from build123d import *

# Parameters (mm, degrees)
SKETCH_1_W                   = 60
SKETCH_1_H                   = 35
EXTRUDE_1_DEPTH              = 5
SKETCH_2_R                   = 2.25
CUT_EXTRUDE_1_DEPTH          = 37.142080737
CUT_EXTRUDE_2_DEPTH          = 37.142080737
SKETCH_5_W                   = 80
SKETCH_5_H                   = 50
EXTRUDE_3_DEPTH              = 10
HOLE_WIZARD_M4_1_D           = 4.5
HOLE_WIZARD_M4_1_CBORE_D     = 8
HOLE_WIZARD_M4_1_CBORE_DEPTH = 4.4
FILLET_1_R                   = 5


with BuildPart() as part:
    # 草图1 → 凸台-拉伸1 (new, symmetric)
    with BuildSketch(Plane(origin=(0, 0, 0), x_dir=(1, 0, 0), z_dir=(0, 1, 0))):
        Rectangle(SKETCH_1_W, SKETCH_1_H)
    extrude(amount=EXTRUDE_1_DEPTH, both=True)

    # 草图2 → 切除-拉伸1 (cut, through all)
    with BuildSketch(Plane.XZ.offset(5)):
        with Locations(Location((-15, 12.5, 0), (0, 0, 270))):
            Circle(SKETCH_2_R)
        with Locations(Location((-15, 2.5, 0), (0, 0, 270))):
            Circle(SKETCH_2_R)
    extrude(amount=-CUT_EXTRUDE_1_DEPTH, mode=Mode.SUBTRACT)

    # 草图3 → 切除-拉伸2 (cut, through all)
    with BuildSketch(Plane.XZ.offset(5)):
        with BuildLine():
            ThreePointArc((-27.188596105, 11.275), (-15, 0.25), (-2.811403895, 11.275))
            ThreePointArc((-2.811403895, 11.275), (-4.825125629, 13.738721733), (-7.288847362, 11.725))
            ThreePointArc((-7.288847362, 11.725), (-15, 4.75), (-22.711152638, 11.725))
            ThreePointArc((-22.711152638, 11.725), (-25.174874371, 13.738721733), (-27.188596105, 11.275))
        make_face()
    extrude(amount=-CUT_EXTRUDE_2_DEPTH, mode=Mode.SUBTRACT)

    # 草图5 → 凸台-拉伸3 (add)
    with BuildSketch(Plane(origin=(30, 0, 0), x_dir=(0, 0, -1), z_dir=(1, 0, 0))):
        Rectangle(SKETCH_5_W, SKETCH_5_H)
    extrude(amount=EXTRUDE_3_DEPTH)

    # M4 六角凹头螺钉的柱形沉头孔1 (through all)
    with Locations(Plane.ZY.offset(-30)):
        with Locations((30, 15), (-30, 15), (-30, -15), (30, -15)):
            CounterBoreHole(HOLE_WIZARD_M4_1_D / 2, HOLE_WIZARD_M4_1_CBORE_D / 2, HOLE_WIZARD_M4_1_CBORE_DEPTH)

    # 圆角1
    fillet_1_edges = [part.edges().sort_by_distance(p)[0] for p in [
        (35, -25, -40),
        (35, 25, -40),
        (35, 25, 40),
        (35, -25, 40),
        (-30, 0, 17.5),
        (-30, 0, -17.5),
    ]]
    fillet(fillet_1_edges, radius=FILLET_1_R)


solid = part.part
Verification items for the finished model (mm, model axes). A direction names the side the tool comes from. Coordinates: 2 decimals unless noted, no trailing zeros. Write each loop counter-clockwise with the first axis right and the second up, starting at its lowest first coordinate (ties: lowest second). Pieces come first, ordered by that corner, then holes. Notation, with made-up numbers: (34.5, 85) -> (81.5, 85) arc R16 cw to (81.5, 93) -> close; hole circle Ø8 at (68, 82). An arc over 180 degrees is marked (long way). One line per item, written item: value. Start each with the question number.
Q1. Thickness scan on L1, parallel to Y at x = 38.35, z = 30; L2, parallel to Y at x = 32.2, z = 30; L3, parallel to Z at x = 36, y = -13.5. Record the ranges inside material, lowest first. Write a range as from..to.
Q2. Cross-section at C-C on x = -15. Enter the section's corners in (y, z), and give its area (3 significant figures).
Q3. Cross-section at B-B on z = 30. Enter the section's corners in (x, y), and give its area (3 significant figures).
Q4. Cross-section at D-D on y = 4. Enter the section's corners in (x, z) (3 decimals), and give its area (3 significant figures).
Q5. Cross-section at A-A on y = -15. Enter the section's corners in (x, z), and give its area (3 significant figures).
Q6. Access from +Z, -Z, +X, -X, +Y, -Y to the whole of each face (thin tool, end or side, straight path). Record for faces 5 (the flat face through (34.4, 13, -28)), 6 (the cylindrical face through (-4.776, -0.07, 13.733)), 7 (the flat face through (0, -5, 0)), 8 (the flat face through (2, 0, 17.5)).
Q7. Mould release check, pull along Y, two halves, no side actions. Record for faces 1 (the flat face through (30, 6, 1)), 2 (the cylindrical face through (32.17, -12.3, 27.05)), 3 (the flat face through (35, -25, 0)), 4 (the cylindrical face through (32.169, 18.966, -30.521)): pulls with the +Y half, pulls with the -Y half, needs draft (parallel to the pull), parting line crosses it, or undercut.
Q8. Go/stop test with flat-tipped pins: P1, Ø6.5, axis at y = -15, z = 30, coming from the -X side; P2, Ø8, axis at x = 7.5, z = -18, coming from the +Y side; P3, Ø1, axis at y = 3.5, z = -22.5, coming from the -X side; P4, Ø2.5, axis at y = 15.5, z = 30.5, coming from the -X side. Record where each tip stops, or that it passes through.
Checked values:
1. L1: y = -25..-17.25, -12.75..12.75, 17.25..25
1. L2: y = -25..-19, -11..11, 19..25
1. L3: z = -40..-31.68, -28.32..28.32, 31.68..40
2. outline: (-5, -17.5) -> (5, -17.5) -> (5, 0.25) -> (-5, 0.25) -> close; (-5, 4.75) -> (5, 4.75) -> (5, 10.25) -> (-5, 10.25) -> close; (-5, 14.75) -> (5, 14.75) -> (5, 17.5) -> (-5, 17.5) -> close
2. area: 260 mm²
3. outline: (30, -25) -> (40, -25) -> (40, -17.25) -> (34.4, -17.25) -> (34.4, -19) -> (30, -19) -> close; (30, -11) -> (34.4, -11) -> (34.4, -12.75) -> (40, -12.75) -> (40, 12.75) -> (34.4, 12.75) -> (34.4, 11) -> (30, 11) -> close; (30, 19) -> (34.4, 19) -> (34.4, 17.25) -> (40, 17.25) -> (40, 25) -> (30, 25) -> close
3. area: 379 mm²
4. outline: (-30, -12.5) arc R5 ccw to (-25, -17.5) -> (30, -17.5) -> (30, -40) -> (40, -40) -> (40, 40) -> (30, 40) -> (30, 17.5) -> (-25, 17.5) arc R5 ccw to (-30, 12.5) -> close; hole (-27.189, 11.275) arc R12.25 ccw to (-2.811, 11.275) arc R2.25 ccw to (-7.289, 11.725) arc R7.75 cw to (-22.711, 11.725) arc R2.25 ccw to start; hole circle Ø4.5 at (-15, 12.5)
4. area: 2,730 mm²
5. outline: (30, -40) -> (40, -40) -> (40, -32.25) -> (34.4, -32.25) -> (34.4, -34) -> (30, -34) -> close; (30, -26) -> (34.4, -26) -> (34.4, -27.75) -> (40, -27.75) -> (40, 27.75) -> (34.4, 27.75) -> (34.4, 26) -> (30, 26) -> close; (30, 34) -> (34.4, 34) -> (34.4, 32.25) -> (40, 32.25) -> (40, 40) -> (30, 40) -> close
5. area: 679 mm²
6. face 5: -X
6. face 6: +Y, -Y
6. face 7: +Z, -Z, -X, -Y
6. face 8: +Z, -X, +Y, -Y
7. face 1: needs draft
7. face 2: undercut
7. face 3: pulls with the -Y half
7. face 4: undercut
8. P1: stops at x = 34.4
8. P2: stops at y = 5
8. P3: stops at x = 30
8. P4: passes through
